from build123d import *

# Parameters (mm, degrees)
BOSS_EXTRUDE1_DEPTH = 123
BOSS_EXTRUDE2_START = -1.2
BOSS_EXTRUDE2_DEPTH = 1.2
FILLET1_R           = 10
FILLET2_R           = 10
CUT_EXTRUDE1_DEPTH  = 353.063005725
SKETCH4_R           = 6.5
CUT_EXTRUDE2_DEPTH  = 353.063005725
SKETCH5_W           = 53
SKETCH5_H           = 220
CUT_EXTRUDE3_DEPTH  = 353.063005725
FILLET3_R           = 10
SKETCH6_R           = 1.75
CUT_EXTRUDE4_DEPTH  = 353.063005725


with BuildPart() as part:
    # Sketch1 → Boss-Extrude1 (new body)
    with BuildSketch(Plane.XY):
        with BuildLine():
            Line((-105, -150.6), (-105, 149.4))
            ThreePointArc((-105, 149.4), (0, 254.4), (105, 149.4))
            Line((105, 149.4), (105, -150.6))
            Line((105, -150.6), (-105, -150.6))
        make_face()
        with BuildLine():
            Line((93.8, -149.4), (-93.8, -149.4))
            ThreePointArc((-93.8, -149.4), (-100.871067812, -146.471067812), (-103.8, -139.4))
            Line((-103.8, -139.4), (-103.8, 149.4))
            ThreePointArc((-103.8, 149.4), (0, 253.2), (103.8, 149.4))
            Line((103.8, 149.4), (103.8, -139.4))
            ThreePointArc((103.8, -139.4), (100.871067812, -146.471067812), (93.8, -149.4))
        make_face(mode=Mode.SUBTRACT)
    extrude(amount=BOSS_EXTRUDE1_DEPTH)

    # Sketch2 → Boss-Extrude2 (add)
    with BuildSketch(Plane.XY.offset(123).offset(BOSS_EXTRUDE2_START)):
        with BuildLine():
            Line((-105, 149.4), (-105, -150.6))
            Line((-105, -150.6), (105, -150.6))
            Line((105, -150.6), (105, 149.4))
            ThreePointArc((105, 149.4), (0, 254.4), (-105, 149.4))
        make_face()
    extrude(amount=BOSS_EXTRUDE2_DEPTH)

    # Fillet1
    fillet1_edges = [part.edges().sort_by_distance(p)[0] for p in [
        (-105, -150.6, 61.5),
    ]]
    fillet(fillet1_edges, radius=FILLET1_R)

    # Fillet2
    fillet2_edges = [part.edges().sort_by_distance(p)[0] for p in [
        (105, -150.6, 61.5),
    ]]
    fillet(fillet2_edges, radius=FILLET2_R)

    # Sketch3 → Cut-Extrude1 (cut, through all)
    with BuildSketch(Plane.ZY.offset(105)):
        with BuildLine():
            Line((2.75, 80.1), (2.75, 82.1))
            ThreePointArc((2.75, 82.1), (5.5, 84.85), (8.25, 82.1))
            Line((8.25, 82.1), (8.25, 80.1))
            ThreePointArc((8.25, 80.1), (5.5, 77.35), (2.75, 80.1))
        make_face()
        with BuildLine():
            Line((2.75, -99.9), (2.75, -97.9))
            ThreePointArc((2.75, -97.9), (5.5, -95.15), (8.25, -97.9))
            Line((8.25, -97.9), (8.25, -99.9))
            ThreePointArc((8.25, -99.9), (5.5, -102.65), (2.75, -99.9))
        make_face()
    extrude(amount=-CUT_EXTRUDE1_DEPTH, mode=Mode.SUBTRACT)

    # Sketch4 → Cut-Extrude2 (cut, through all)
    with BuildSketch(Plane.ZY.offset(105)):
        with Locations(Location((11.5, 111.4, 0), (0, 0, 270))):
            Circle(SKETCH4_R)
    extrude(amount=-CUT_EXTRUDE2_DEPTH, mode=Mode.SUBTRACT)

    # Sketch5 → Cut-Extrude3 (cut, through all)
    with BuildSketch(Plane(origin=(105, 0, 0), x_dir=(0, 0, -1), z_dir=(1, 0, 0))):
        with Locations((-68.5, -0.6)):
            Rectangle(SKETCH5_W, SKETCH5_H)
    extrude(amount=-CUT_EXTRUDE3_DEPTH, mode=Mode.SUBTRACT)

    # Fillet3
    fillet3_edges = [part.edges().sort_by_distance(p)[0] for p in [
        (-104.4, 109.4, 95),
        (-104.4, 109.4, 42),
        (-104.4, -110.6, 42),
        (-104.4, -110.6, 95),
        (104.4, 109.4, 95),
        (104.4, 109.4, 42),
        (104.4, -110.6, 42),
        (104.4, -110.6, 95),
    ]]
    fillet(fillet3_edges, radius=FILLET3_R)

    # Sketch6 → Cut-Extrude4 (cut, through all)
    with BuildSketch(Plane(origin=(105, 0, 0), x_dir=(0, 0, -1), z_dir=(1, 0, 0))):
        with Locations(Location((-37, 109.4, 0), (0, 0, 90))):
            Circle(SKETCH6_R)
        with Locations(Location((-37, -0.6, 0), (0, 0, 90))):
            Circle(SKETCH6_R)
        with Locations(Location((-37, -110.6, 0), (0, 0, 90))):
            Circle(SKETCH6_R)
        with Locations(Location((-100, -110.6, 0), (0, 0, 90))):
            Circle(SKETCH6_R)
        with Locations(Location((-100, -0.6, 0), (0, 0, 90))):
            Circle(SKETCH6_R)
        with Locations(Location((-100, 109.4, 0), (0, 0, 90))):
            Circle(SKETCH6_R)
    extrude(amount=-CUT_EXTRUDE4_DEPTH, mode=Mode.SUBTRACT)


solid = part.part
Could you check a few things on this model? Use its own coordinates, in mm. A direction names the side the tool comes from. Round coordinates to 2 decimals unless told otherwise and drop trailing zeros. Order: outer loops, then holes, each group sorted by start corner. A loop starts at its lowest first (then second) coordinate and runs counter-clockwise, first axis right, second up. Notation, with made-up numbers: M -14,27.25 L 27,27.25 A16 ccw 27,33.25 Z; hole C -34,48 d11. An arc over 180 degrees is marked long. One line per item, written item: value.
(1) I need wall thicknesses on line 1 along Z through (x, y) = (-104.7, -0.6); line 2 along X through (y, z) = (-106.5, 110.5); line 3 along Z through (x, y) = (-104, 0). Which ranges of each line are inside material? Lowest first, please. Write a range as from..to.
Ans:
line 1: z = 0..35.25, 38.75..42, 95..98.25, 101.75..123
line 2: x = -105..-103.8, 103.8..105
line 3: z = 0..35.36, 38.64..42, 95..98.36, 101.64..123
(2) Imagine slicing it at A-A (y = -29). Write out the boundary of the cut face in (x, z), and give its area (3 significant figures).
Ans:
outline: M -105,0 L -103.8,0 L -103.8,42 L -105,42 Z; M -105,95 L -103.8,95 L -103.8,121.8 L 103.8,121.8 L 103.8,95 L 105,95 L 105,123 L -105,123 Z; M 103.8,0 L 105,0 L 105,42 L 103.8,42 Z
area: 417 mm^2
(3) Which directions (+Z, -Z, +X, -X, +Y, -Y) give clear straight access to the entire face, cutting with the end or side of a thin tool? Please do faces 1 (the cylindrical face through (-104.41, 106.55, 91.99)), 2 (the flat face through (1, -149.4, 60)), 3 (the cylindrical face through (-2.309, 254.375, 60.639)).
Ans:
face 1: +X, -X
face 2: -Z
face 3: +Z, -Z, +Y
(4) Imagine slicing it at D-D (x = 0). Write out the boundary of the cut face in (y, z), and give its area (3 significant figures).
Ans:
outline: M -150.6,0 L -149.4,0 L -149.4,121.8 L 253.2,121.8 L 253.2,0 L 254.4,0 L 254.4,123 L -150.6,123 Z
area: 778 mm^2
(5) Imagine slicing it at B-B (z = 115). Write out the boundary of the cut face in (x, y).
Ans:
outline: M -105,-140.6 A10 ccw -95,-150.6 L 95,-150.6 A10 ccw 105,-140.6 L 105,149.4 A105 ccw -105,149.4 Z; hole M -103.8,-139.4 A10 ccw -93.8,-149.4 L 93.8,-149.4 A10 ccw 103.8,-139.4 L 103.8,149.4 A103.8 ccw -103.8,149.4 Z
(6) Imagine slicing it at C-C (y = -117). Write out the boundary of the cut face in (x, z), and give its area (3 significant figures).
Ans:
outline: M -105,0 L -103.8,0 L -103.8,121.8 L 103.8,121.8 L 103.8,0 L 105,0 L 105,123 L -105,123 Z
area: 544 mm^2
(7) I'm going to push flat-ended pins straight in: P1, Ø1.3, axis at x = 104.5, y = 38, coming from the -Z side; P2, Ø1, axis at x = 104, z = 69.5, coming from the -Y side; P3, Ø4, axis at x = -22.5, z = 18.5, coming from the +Y side; P4, Ø10, axis at x = 17, y = -35.5, coming from the -Z side. Where does each tip first touch, or does it pass through?
Ans:
P1: stops at z = 0
P2: stops at y = -145.87
P3: stops at y = 252.38
P4: stops at z = 121.8
(8) If we mould it in two halves opening along Z, with no side actions, what happens to faces 4 (the cylindrical face through (104.39, -107.75, 91.99)), 5 (the flat face through (1, 55, 123)), 6 (the flat face through (105, 6, 33))? For each: released by +Z, released by -Z, zero draft, split by the parting line, or undercut.
Ans:
face 4: undercut
face 5: released by +Z
face 6: zero draft
